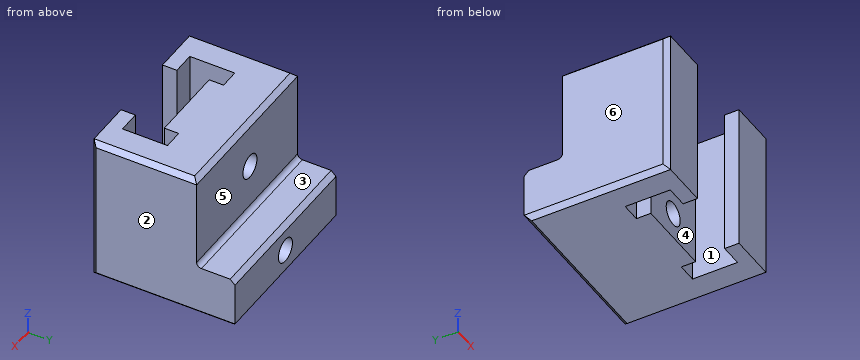
from build123d import *

# Parameters (mm, degrees)
BOSS_EXTRUDE1_START   = -14
BOSS_EXTRUDE1_DEPTH   = 15.5
SKETCH2_W             = 10
SKETCH2_H             = 4
CUT_EXTRUDE1_DEPTH    = 37.060227398
M3_TAPPED_HOLE1_D     = 2.5
M3_TAPPED_HOLE1_DEPTH = 8.5
M3_TAPPED_HOLE1_TIP   = 0.751075774
M3_TAPPED_HOLE2_D     = 2.5
CHAMFER1_SIZE         = 0.5
FILLET1_R             = 0.5


with BuildPart() as part:
    # Sketch1 → Boss-Extrude1 (new body)
    with BuildSketch(Plane.XY.offset(BOSS_EXTRUDE1_START)):
        Polygon((-3.7, -3.2), (-3.7, -4.7), (-9, -4.7), (-9, 10.3), (9, 10.3), (9, -4.7), (3.7, -4.7), (3.7, -3.2), (6, -3.2), (6, 1.5), (4, 1.5), (4, 0), (0, 0), (-4, 0), (-4, 1.5), (-6, 1.5), (-6, -3.2), align=None)
    extrude(amount=-BOSS_EXTRUDE1_DEPTH)

    # Sketch2 → Cut-Extrude1 (cut, through all)
    with BuildSketch(Plane(origin=(9, 0, 0), x_dir=(0, 0, -1), z_dir=(1, 0, 0))):
        with Locations((19, 8.3)):
            Rectangle(SKETCH2_W, SKETCH2_H)
    extrude(amount=-CUT_EXTRUDE1_DEPTH, mode=Mode.SUBTRACT)

    # M3 Tapped Hole1
    with Locations(Plane(origin=(0, 6.3, 0), x_dir=(1, 0, 0), z_dir=(0, 1, 0))):
        with Locations((-0.5, 19)):
            Hole(M3_TAPPED_HOLE1_D / 2, depth=M3_TAPPED_HOLE1_DEPTH)
            with Locations((0, 0, -(M3_TAPPED_HOLE1_DEPTH + M3_TAPPED_HOLE1_TIP / 2))):  # 118° drill point
                Cone(0, M3_TAPPED_HOLE1_D / 2, M3_TAPPED_HOLE1_TIP, mode=Mode.SUBTRACT)

    # M3 Tapped Hole2 (through all)
    with Locations(Plane(origin=(0, 10.3, 0), x_dir=(1, 0, 0), z_dir=(0, 1, 0))):
        with Locations((0, 26.75)):
            Hole(M3_TAPPED_HOLE2_D / 2)

    # Chamfer1
    chamfer1_edges = [part.edges().sort_by_distance(p)[0] for p in [
        (0, 10.3, -29.5),
        (-9, 2.8, -29.5),
        (-9, 0.8, -14),
        (9, 0.8, -14),
        (-9, -4.7, -21.75),
        (9, -4.7, -21.75),
        (0, 6.3, -14),
        (0, 10.3, -24),
        (9, 2.8, -29.5),
    ]]
    chamfer(chamfer1_edges, length=CHAMFER1_SIZE)

    # Fillet1
    fillet1_edges = [part.edges().sort_by_distance(p)[0] for p in [
        (0, 6.3, -24),
    ]]
    fillet(fillet1_edges, radius=FILLET1_R)


solid = part.part
CAD build for the part. Positions are in the model's coordinates, mm. Face numbers are marked on the shaded views. A direction names the side the tool comes from. Round coordinates to 2 decimals unless told otherwise and drop trailing zeros. Loops run counter-clockwise (first coordinate to the right, second up) from the corner with the lowest first, then second, coordinate; pieces in that order, holes last.
(1) Cut at B-B (z = -19). Give the cut face in (x, y).
(2) Two-plate mould, pull along X, no slides. Class the marked faces 4, 5 and 6: +X half, -X half, draft (parallel to the pull), parting line (faces both ways), or undercut.
(3) Cut at D-D (z = -24.25). Give the cut face in (x, y).
(4) Drop flat-ended pins along their axis: pin 1 (3 mm diameter, centred on x = 1.5, z = -20, fed in from -Y); pin 2 (1.5 mm diameter, centred on x = 1, y = 8, fed in from +Z); pin 3 (1.2 mm diameter, centred on x = -5, z = -18, fed in from +Y). Give the stop position or say it passes through.
(5) Which spindle directions (+Z, -Z, +X, -X, +Y, -Y) get a long thin tool onto all of the face, cutting with end or side? Do the marked faces 1, 2 and 3. Say none if no direction does.
(6) Cut at A-A (y = -2.5). Give the cut face in (x, z).
(7) Wall check: line 1 along X through (y, z) = (-3.25, -14.75); line 2 along Y through (x, z) = (-4.5, -27.25); line 3 along X through (y, z) = (-1.75, -22). Give the ranges that are in metal, low to high.
(8) Cut at C-C (y = 9). Give the cut face in (x, z), plus the area to 3 significant figures.
Findings below:
1. outline: (-9, -4.2) - (-8.5, -4.7) - (-3.7, -4.7) - (-3.7, -3.2) - (-6, -3.2) - (-6, 1.5) - (-4, 1.5) - (-4, 0) - (-1.75, 0) - (-1.75, 6.3) - (-9, 6.3) - close; (0.75, 0) - (4, 0) - (4, 1.5) - (6, 1.5) - (6, -3.2) - (3.7, -3.2) - (3.7, -4.7) - (8.5, -4.7) - (9, -4.2) - (9, 6.3) - (0.75, 6.3) - close
2. face 4: undercut
2. face 5: draft
2. face 6: -X half
3. outline: (-9, -4.2) - (-8.5, -4.7) - (-3.7, -4.7) - (-3.7, -3.2) - (-6, -3.2) - (-6, 1.5) - (-4, 1.5) - (-4, 0) - (4, 0) - (4, 1.5) - (6, 1.5) - (6, -3.2) - (3.7, -3.2) - (3.7, -4.7) - (8.5, -4.7) - (9, -4.2) - (9, 10.05) - (-9, 10.05) - close
4. pin 1: stops at y = 0
4. pin 2: stops at z = -24
4. pin 3: stops at y = 6.3
5. face 1: +Z, -Z
5. face 2: +Z, -Z, +X, +Y, -Y
5. face 3: +Z, +X, -X, +Y
6. outline: (-9, -29) - (-8.5, -29.5) - (-6, -29.5) - (-6, -14) - (-8.5, -14) - (-9, -14.5) - close; (6, -29.5) - (8.5, -29.5) - (9, -29) - (9, -14.5) - (8.5, -14) - (6, -14) - close
7. line 1: x = -9 to -3.7, 3.7 to 9
7. line 2: y = -4.7 to -3.2, 1.5 to 10.3
7. line 3: x = -9 to -6, 6 to 9
8. outline: (-9, -29) - (-8.5, -29.5) - (8.5, -29.5) - (9, -29) - (9, -24) - (-9, -24) - close; hole circle Ø2.5 at (0, -26.75)
8. area: 93.8 mm2
